Could you check a few things on this model? Use its own coordinates, in mm. A direction names the side the tool comes from. Round coordinates to 2 decimals unless told otherwise and drop trailing zeros. Loops run counter-clockwise (first coordinate to the right, second up) from the corner with the lowest first, then second, coordinate; pieces in that order, holes last. Notation, with made-up numbers: (81.25, 5.25) - (127.25, 5.25) arc R23 cw to (127.25, 13.25) - close; hole circle Ø11 at (67, 12.25). An arc over 180 degrees is marked (long way). Use one line per item in the form item = value.
```python
from build123d import *

# Parameters (mm, degrees)
SKETCH_1_W                   = 35
SKETCH_1_H                   = 4
EXTRUDE_1_DEPTH              = 40
SKETCH_2_W                   = 7
SKETCH_2_H                   = 40
EXTRUDE_2_DEPTH              = 12
HOLE_WIZARD_M3_1_D           = 2.5
HOLE_WIZARD_M3_1_DEPTH       = 7.5
HOLE_WIZARD_M3_1_CBORE_D     = 3
HOLE_WIZARD_M3_1_CBORE_DEPTH = 6
HOLE_WIZARD_M3_1_TIP         = 0.751075774
SKETCH_9_W                   = 7
SKETCH_9_H                   = 40
EXTRUDE_3_DEPTH              = 10
SKETCH_14_W                  = 40
SKETCH_14_H                  = 3.5
CUT_EXTRUDE_5_DEPTH          = 55.083269132
SKETCH_15_W                  = 2
SKETCH_15_H                  = 2
CUT_EXTRUDE_6_DEPTH          = 54.546708582
EXTRUDE_5_DEPTH              = 2
CUT_EXTRUDE_7_DEPTH          = 54.546708582
FILLET_1_R                   = 1
CUT_EXTRUDE_8_DEPTH          = 55.177947543


with BuildPart() as part:
    # 草图1 → 拉伸1 (new body)
    with BuildSketch(Plane.XY):
        with Locations((17.5, 2)):
            Rectangle(SKETCH_1_W, SKETCH_1_H)
    extrude(amount=EXTRUDE_1_DEPTH)

    # 草图2 → 拉伸2 (add)
    with BuildSketch(Plane(origin=(0, 4, 0), x_dir=(-1, 0, 0), z_dir=(0, 1, 0))):
        with Locations((-3.5, 20)):
            Rectangle(SKETCH_2_W, SKETCH_2_H)
    extrude(amount=-EXTRUDE_2_DEPTH)

    # M3 螺纹孔1
    with Locations(Plane.XZ.offset(8)):
        with Locations((3.5, 3), (3.5, 37)):
            CounterBoreHole(HOLE_WIZARD_M3_1_D / 2, HOLE_WIZARD_M3_1_CBORE_D / 2, HOLE_WIZARD_M3_1_CBORE_DEPTH, depth=HOLE_WIZARD_M3_1_DEPTH)
            with Locations((0, 0, -(HOLE_WIZARD_M3_1_DEPTH + HOLE_WIZARD_M3_1_TIP / 2))):  # 118° drill point
                Cone(0, HOLE_WIZARD_M3_1_D / 2, HOLE_WIZARD_M3_1_TIP, mode=Mode.SUBTRACT)

    # 草图9 → 拉伸3 (add)
    with BuildSketch(Plane.XZ):
        with Locations((31.5, 20)):
            Rectangle(SKETCH_9_W, SKETCH_9_H)
    extrude(amount=EXTRUDE_3_DEPTH)

    # 草图14 → 切除-拉伸5 (cut, through all)
    with BuildSketch(Plane(origin=(35, 0, 0), x_dir=(0, 0, -1), z_dir=(1, 0, 0))):
        with Locations((-20, -8.25)):
            Rectangle(SKETCH_14_W, SKETCH_14_H)
    extrude(amount=-CUT_EXTRUDE_5_DEPTH, mode=Mode.SUBTRACT)

    # 草图15 → 切除-拉伸6 (cut, through all)
    with BuildSketch(Plane.ZY):
        with Locations((1, 3)):
            Rectangle(SKETCH_15_W, SKETCH_15_H)
        with Locations((39, 3)):
            Rectangle(SKETCH_15_W, SKETCH_15_H)
    extrude(amount=-CUT_EXTRUDE_6_DEPTH, mode=Mode.SUBTRACT)

    # 草图17 → 拉伸5 (add)
    with BuildSketch(Plane(origin=(0, 4, 0), x_dir=(1, 0, 0), z_dir=(0, 1, 0))):
        Polygon((-20, -2), (35, -2), (35, -8), (10, -8), (10, -32), (35, -32), (35, -38), (-20, -38), align=None)
    extrude(amount=EXTRUDE_5_DEPTH)

    # 草图18 → 切除-拉伸7 (cut, through all)
    with BuildSketch(Plane.ZY):
        Polygon((31.15, -4.508141571), (28.85, -4.508141571), (27.7, -6.5), (28.85, -8.491858429), (31.15, -8.491858429), (32.3, -6.5), align=None)
    cut_extrude_7 = extrude(amount=-CUT_EXTRUDE_7_DEPTH, mode=Mode.SUBTRACT)

    # 镜向1: 切除-拉伸7 across plane
    add(cut_extrude_7.mirror(Plane(origin=(0, 0, 20), x_dir=(1, 0, 0), z_dir=(0, 0, -1))), mode=Mode.SUBTRACT)

    # 圆角1
    fillet_1_edges = [part.edges().sort_by_distance(p)[0] for p in [
        (10, 5, 32),
        (10, 5, 8),
    ]]
    fillet(fillet_1_edges, radius=FILLET_1_R)

    # 草图20 → 切除-拉伸8 (cut, through all)
    with BuildSketch(Plane.XZ.offset(-4)):
        with BuildLine():
            Line((-15, 22.5), (-5, 22.5))
            ThreePointArc((-5, 22.5), (-2.5, 20), (-5, 17.5))
            Line((-5, 17.5), (-15, 17.5))
            ThreePointArc((-15, 17.5), (-17.5, 20), (-15, 22.5))
        make_face()
    extrude(amount=-CUT_EXTRUDE_8_DEPTH, mode=Mode.SUBTRACT)


solid = part.part
```
1. For P1, Ø2.5, axis at x = 3, z = 9.5, coming from the -Y side; P2, Ø2, axis at x = 15.5, y = 3.5, coming from the +Z side; P3, Ø4.5, axis at x = 11.5, y = 5, coming from the -Z side, each with a flat end and sliding along its axis, tell me the tip position at first contact or that it passes through.
Solution:
P1 = -5.55
P2 = 38
P3 = 2
2. Please list where these lines run through material, in increasing order: line 1 along Z through (x, y) = (3.5, -1.1); line 2 along X through (y, z) = (-1.3, 37); line 3 along Z through (x, y) = (3.5, -4.25).
Solution:
line_1 = 0 to 1.75, 4.25 to 35.75, 38.25 to 40
line_2 = 0 to 2.25, 4.75 to 7, 28 to 35
line_3 = 0 to 1.5, 4.5 to 35.5, 38.5 to 40
3. If we section it at C-C, the plane z = 33.5: Write out the boundary of the cut face in (x, y).
Solution:
outline = (-20, 4) - (0, 4) - (0, -6.5) - (7, -6.5) - (7, 0) - (28, 0) - (28, -6.5) - (35, -6.5) - (35, 6) - (-20, 6) - close
4. If we section it at A-A, the plane z = 18.5: Write out the boundary of the cut face in (x, y), plus the area to 3 significant figures.
Solution:
outline = (-20, 4) - (-17, 4) - (-17, 6) - (-20, 6) - close; (-3, 4) - (0, 4) - (0, -6.5) - (7, -6.5) - (7, 0) - (28, 0) - (28, -6.5) - (35, -6.5) - (35, 4) - (10, 4) - (10, 6) - (-3, 6) - close
area = 263 mm^2
5. If we section it at B-B, the plane x = -12: Write out the boundary of the cut face in (y, z).
Solution:
outline = (4, 2) - (6, 2) - (6, 17.5) - (4, 17.5) - close; (4, 22.5) - (6, 22.5) - (6, 38) - (4, 38) - close
6. If we section it at D-D, the plane x = 23: Write out the boundary of the cut face in (y, z).
Solution:
outline = (0, 0) - (2, 0) - (2, 2) - (6, 2) - (6, 8) - (4, 8) - (4, 32) - (6, 32) - (6, 38) - (2, 38) - (2, 40) - (0, 40) - close
7. On a 3-axis mill with a long thin cutter (end or side, diameter ignored), from which of +Z, -Z, +X, -X, +Y, -Y can I reach the whole of each face in a straight line? I mean faces 4 (the face through (4, -6.5, 5)), 5 (the face through (-10, 4, 24)), 6 (the face through (31.451, -5.518, 8.267)), 7 (the face through (-2.5, 5, 20.1)), 8 (the face through (17, 0, 20)). Say none if no direction works.
Solution:
face_4 = +Z, -Z, +X, -X, -Y
face_5 = +Z, -Z, -X, -Y
face_6 = +X, -X, -Y
face_7 = +Y, -Y
face_8 = +Z, -Z, -Y
8. We'd pull the mould along X, two halves only. Please class faces 1 (the face through (31.451, -5.49, 11.717)), 2 (the face through (-10, 5, 17.5)), 3 (the face through (4.19, -4.28, 35.67)): +X half, -X half, draft (parallel to the pull), parting line (faces both ways), or undercut.
Solution:
face_1 = draft
face_2 = undercut
face_3 = undercut
